from build123d import *

# Parameters (mm, degrees)
SKETCH1_R           = 1.5
BOSS_EXTRUDE1_DEPTH = 3
FILLET1_R           = 3


with BuildPart() as part:
    # Sketch1 → Boss-Extrude1 (new body)
    with BuildSketch(Plane(origin=(0, 0, 0), x_dir=(1, 0, 0), z_dir=(0, 1, 0))):
        with BuildLine():
            ThreePointArc((3.16227766, 1.5), (-3.5, 0), (3.16227766, -1.5))
            Line((3.16227766, -1.5), (27.83772234, -1.5))
            ThreePointArc((27.83772234, -1.5), (34.5, 0), (27.83772234, 1.5))
            Line((27.83772234, 1.5), (3.16227766, 1.5))
        make_face()
        with Locations(Location((0, 0, 0), (0, 0, 270))):
            Circle(SKETCH1_R, mode=Mode.SUBTRACT)
        with Locations(Location((31, 0, 0), (0, 0, 270))):
            Circle(SKETCH1_R, mode=Mode.SUBTRACT)
    extrude(amount=BOSS_EXTRUDE1_DEPTH)

    # Fillet1
    fillet1_edges = [part.edges().sort_by_distance(p)[0] for p in [
        (27.83772234, 1.5, 1.5),
        (3.16227766, 1.5, 1.5),
        (3.16227766, 1.5, -1.5),
        (27.83772234, 1.5, -1.5),
    ]]
    fillet(fillet1_edges, radius=FILLET1_R)


solid = part.part
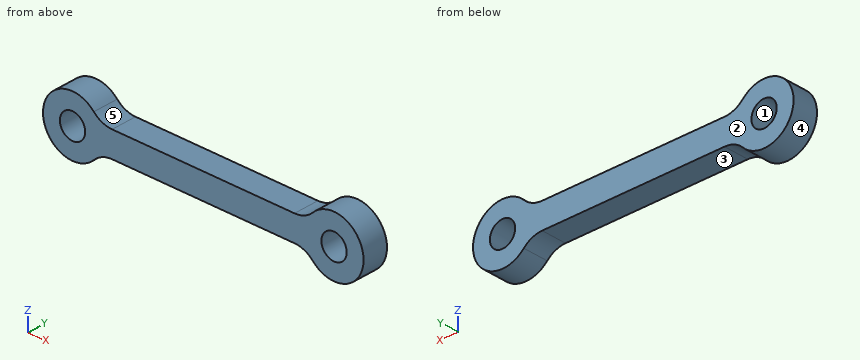
For this review, take the finished solid that the model builds, in its own axes (mm). Face numbers are marked on the shaded views. A direction names the side the tool comes from. Give positions to 0.01 mm unless a question says otherwise; leave off trailing zeros. Loops run counter-clockwise (first coordinate to the right, second up) from the corner with the lowest first, then second, coordinate; pieces in that order, holes last. Notation, with made-up numbers: (60.5, -24) -> (116.5, -24) arc R23 cw to (116.5, -2) -> close; hole circle Ø6 at (81, 8). An arc over 180 degrees is marked (long way). One line per question, with ' | ' between items.
1) We need section D-D (z = 3). Write out the cut boundary in (x, y).
Resolved:
outline: (-1.8, 0) -> (1.8, 0) -> (1.8, 3) -> (-1.8, 3) -> close; (29.2, 0) -> (32.8, 0) -> (32.8, 3) -> (29.2, 3) -> close
2) We need section C-C (y = 0.45). Write out the cut boundary in (x, z), plus the area to 3 significant figures.
Resolved:
outline: (2.53, -2.42) arc R3 cw to (4.69, -1.5) -> (26.31, -1.5) arc R3 cw to (28.47, -2.42) arc R3.5 ccw (long way) to (28.47, 2.42) arc R3 cw to (26.31, 1.5) -> (4.69, 1.5) arc R3 cw to (2.53, 2.42) arc R3.5 ccw (long way) to start; hole circle Ø3 at (0, 0); hole circle Ø3 at (31, 0) | area: 137 mm2
3) The part is to be moulded in two halves that separate along X. For the marked faces 1 and 2, say which applies: +X half, -X half, draft (parallel to the pull), parting line (faces both ways), or undercut.
Resolved:
face 1: undercut | face 2: draft
4) To check wall thickness, follow probe 1 along X at (y, z) = (1.15, 0); probe 2 along X at (y, z) = (0.75, -1.25); probe 3 along Z at (x, y) = (9, 1.85). State the ranges of each line that lie inside material, in increasing order.
Resolved:
probe 1: x = -3.5 to -1.5, 1.5 to 29.5, 32.5 to 34.5 | probe 2: x = -3.27 to -0.83, 0.83 to 30.17, 31.83 to 34.27 | probe 3: z = -1.5 to 1.5
5) Insertion check: pin 1 Ø1 at (x, z) = (13, -3) entering from -Y; pin 2 Ø1.5 at (x, y) = (18.5, 2) entering from -Z; pin 3 Ø1.5 at (x, y) = (28, 1) entering from +Z; pin 4 Ø3.5 at (x, z) = (31, 0) entering from +Y. Each pin has a flat end and moves straight along its axis. Give the tip position at first contact, or say it passes through.
Resolved:
pin 1: passes through | pin 2: stops at z = -1.5 | pin 3: stops at z = 2.68 | pin 4: stops at y = 3
6) For the marked faces 3, 4 and 5, list the 3-axis set-ups (+Z, -Z, +X, -X, +Y, -Y) from which the entire face can be reached by the end or side of a thin tool; tool diameter is ignored.
Resolved:
face 3: -Z, +Y, -Y | face 4: +Y, -Y | face 5: +Z, +Y, -Y
7) We need section A-A (x = 31). Write out the cut boundary in (y, z), plus the area to 3 significant figures.
Resolved:
outline: (0, -3.5) -> (3, -3.5) -> (3, -1.5) -> (0, -1.5) -> close; (0, 1.5) -> (3, 1.5) -> (3, 3.5) -> (0, 3.5) -> close | area: 12.0 mm2
8) We need section B-B (z = 0). Write out the cut boundary in (x, y).
Resolved:
outline: (-3.5, 0) -> (-1.5, 0) -> (-1.5, 3) -> (-3.5, 3) -> close; (1.5, 0) -> (29.5, 0) -> (29.5, 3) -> (1.5, 3) -> close; (32.5, 0) -> (34.5, 0) -> (34.5, 3) -> (32.5, 3) -> close
